```python
from build123d import *


with BuildPart() as part:
    # Sketch1 → Revolve1 (revolve)
    with BuildSketch(Plane.XY):
        Polygon((828.372635386, 15), (808.372635386, 15), (808.372635386, 12), (804.372635386, 12), (804.372635386, 15), (802.372635386, 15), (798.372635386, 19), (742.072635386, 19), (742.072635386, 25), (738.072635386, 29), (684.582635386, 29), (666.582635386, 29), (513.022635386, 29), (513.022635386, 0), (830.872635386, 0), (830.872635386, 12.5), align=None)
    revolve(axis=Axis((838.372635386, 0, 0), (-1, 0, 0)))


solid = part.part
```
Could you check a few things on this model? Use its own coordinates, in mm. A direction names the side the tool comes from. Coordinates: 2 decimals unless noted, no trailing zeros. Write each loop counter-clockwise with the first axis right and the second up, starting at its lowest first coordinate (ties: lowest second). Pieces come first, ordered by that corner, then holes. Notation, with made-up numbers: (-16, -30.5) -> (4, -30.5) arc R18 ccw to (4, -13.5) -> close; hole circle Ø8 at (-6.5, 43.25). An arc over 180 degrees is marked (long way). One line per question, with ' | ' between items. Start each with the question number.
1. Will these pins go through, and if not, where does the flat tip stop? P1, Ø6, axis at x = 789, y = 10, coming from the +Z side; P2, Ø1, axis at x = 632, y = 17.5, coming from the -Z side; P3, Ø1, axis at x = 766.5, z = 5, coming from the -Y side.
2. If we section it at C-C (x = 665): Please give me the cut outline in (y, z), and give its area (3 significant figures).
3. For faces 1 (the face through (808.373, -7, -10)), 2 (the face through (513.023, 0, 0)), 3 (the face through (742.073, 4, -19)), which set-ups out of +Z, -Z, +X, -X, +Y, -Y let a thin tool reach every point of the face, with its end or its side?
4. Please list where these lines run through material, in increasing order: line 1 along X through (y, z) = (-18, 12.5); line 2 along Y through (x, z) = (574, 1); line 3 along X through (y, z) = (-7, 11).
5. Thinking about a two-plate mould opening in X: for faces 4 (the face through (804.373, 7, -10)), 5 (the face through (806.34, -11.99, -0.53)), 6 (the face through (803.359, -14.985, -0.66)), 7 (the face through (830.72, -12.64, -0.56)), which applies, pulls with the +X half, pulls with the -X half, needs draft (parallel to the pull), parting line crosses it, or undercut?
6. If we section it at A-A (z = 0): Please give me the cut outline in (x, y), and give its area (3 significant figures).
7. If we section it at D-D (x = 762.5): Please give me the cut outline in (y, z).
Return value:
1) P1: stops at z = 17.66 | P2: stops at z = -23.49 | P3: stops at y = -18.46
2) outline: circle Ø58 at (0, 0) | area: 2,640 mm²
3) face 1: none | face 2: +Z, -Z, -X, +Y, -Y | face 3: +X
4) line 1: x = 513.02 to 742.07 | line 2: y = -28.98 to 28.98 | line 3: x = 513.02 to 804.37, 808.37 to 830.33
5) face 4: undercut | face 5: undercut | face 6: needs draft | face 7: pulls with the +X half
6) outline: (513.02, -29) -> (738.07, -29) -> (742.07, -25) -> (742.07, -19) -> (798.37, -19) -> (802.37, -15) -> (804.37, -15) -> (804.37, -12) -> (808.37, -12) -> (808.37, -15) -> (828.37, -15) -> (830.87, -12.5) -> (830.87, 12.5) -> (828.37, 15) -> (808.37, 15) -> (808.37, 12) -> (804.37, 12) -> (804.37, 15) -> (802.37, 15) -> (798.37, 19) -> (742.07, 19) -> (742.07, 25) -> (738.07, 29) -> (513.02, 29) -> close | area: 16,400 mm²
7) outline: circle Ø38 at (0, 0)
